Geometry check sheet. Reference: the model listing, model coordinates, mm. Face numbers are marked on the shaded views. Round coordinates to 2 decimals unless told otherwise and drop trailing zeros. Loops run counter-clockwise (first coordinate to the right, second up) from the corner with the lowest first, then second, coordinate; pieces in that order, holes last. Notation, with made-up numbers: (11.5, 37.25) -> (29.5, 37.25) arc R7 cw to (29.5, 47.25) -> close; hole circle Ø10 at (18.25, -20.75). An arc over 180 degrees is marked (long way). Use one line per item in the form item = value.
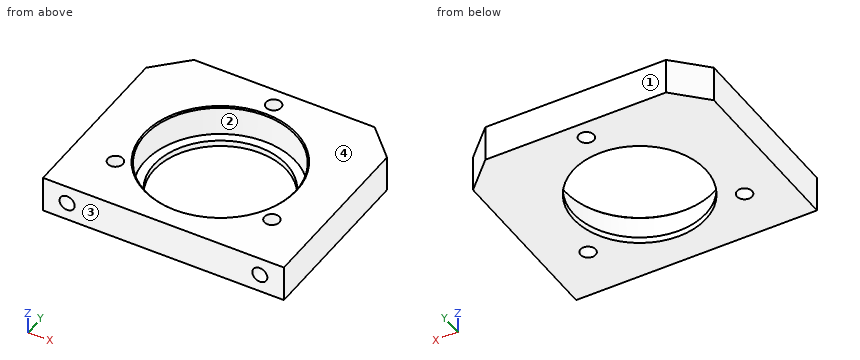
from build123d import *

# Parameters (mm, degrees)
SKETCH_1_R             = 11
EXTRUDE_1_DEPTH        = 6
SKETCH_2_R             = 12.5
CUT_EXTRUDE_1_DEPTH    = 5
HOLE_WIZARD_M3_1_D     = 2.5
HOLE_WIZARD_M3_2_D     = 2.5
HOLE_WIZARD_M3_2_DEPTH = 6
HOLE_WIZARD_M3_2_TIP   = 0.751075774
CHAMFER_1_SIZE         = 0.2


with BuildPart() as part:
    # 草图1 → 凸台-拉伸1 (new body)
    with BuildSketch(Plane.XY):
        Polygon((-20, -16), (20, -16), (20, 13), (15, 18), (-15, 18), (-20, 13), align=None)
        Circle(SKETCH_1_R, mode=Mode.SUBTRACT)
    extrude(amount=EXTRUDE_1_DEPTH)

    # 草图2 → 切除-拉伸1 (cut)
    with BuildSketch(Plane.XY.offset(6)):
        Circle(SKETCH_2_R)
    extrude(amount=-CUT_EXTRUDE_1_DEPTH, mode=Mode.SUBTRACT)

    # M3 螺纹孔1 (through all)
    with Locations(Plane(origin=(0, 15.005632156, 6), x_dir=(1, 0, 0), z_dir=(0, 0, 1))):
        with Locations((0, 0), (-12.990381057, -22.505632156), (12.990381057, -22.505632156)):
            Hole(HOLE_WIZARD_M3_1_D / 2)

    # M3 螺纹孔2
    with Locations(Plane(origin=(-16, -16, 3), x_dir=(0, 0, -1), z_dir=(0, -1, 0))):
        with Locations((0, 0), (0, 32)):
            Hole(HOLE_WIZARD_M3_2_D / 2, depth=HOLE_WIZARD_M3_2_DEPTH)
            with Locations((0, 0, -(HOLE_WIZARD_M3_2_DEPTH + HOLE_WIZARD_M3_2_TIP / 2))):  # 118° drill point
                Cone(0, HOLE_WIZARD_M3_2_D / 2, HOLE_WIZARD_M3_2_TIP, mode=Mode.SUBTRACT)

    # 倒角1
    chamfer_1_edges = [part.edges().sort_by_distance(p)[0] for p in [
        (-12.5, 0, 6),
    ]]
    chamfer(chamfer_1_edges, length=CHAMFER_1_SIZE)


solid = part.part
1. Gauge pin test, flat ends, axial feed: pin 1 (2 mm diameter, centred on x = -16, z = 3, fed in from -Y); pin 2 (1.5 mm diameter, centred on x = 16, z = 3, fed in from +Y). Record the tip position at first contact, or that the pin passes through.
Return value:
pin_1 = -9.85
pin_2 = 17.75
2. Section check A-A (z = 5.35). Record the boundary of the cut face in (x, y), then the cut area to 3 significant figures.
Return value:
outline = (-20, -16) -> (20, -16) -> (20, 13) -> (15, 18) -> (-15, 18) -> (-20, 13) -> close; hole circle Ø2.5 at (-12.99, -7.5); hole circle Ø25 at (0, 0); hole circle Ø2.5 at (0, 15.01); hole circle Ø2.5 at (12.99, -7.5)
area = 829 mm2
3. Section check C-C (z = 0.45). Record the boundary of the cut face in (x, y), then the cut area to 3 significant figures.
Return value:
outline = (-20, -16) -> (20, -16) -> (20, 13) -> (15, 18) -> (-15, 18) -> (-20, 13) -> close; hole circle Ø2.5 at (-12.99, -7.5); hole circle Ø22 at (0, 0); hole circle Ø2.5 at (0, 15.01); hole circle Ø2.5 at (12.99, -7.5)
area = 940 mm2
4. Section check B-B (y = -7.5). Count the separate pieces of the cut face and the enclosed holes in it, then the cut area to 3 significant figures.
Return value:
separate_pieces = 4
enclosed_holes = 0
area = 93.9 mm2
5. Mould release check, pull along Y, two halves, no side actions. Record for the marked faces 1, 2, 3 and 4: released by +Y, released by -Y, zero draft, split by the parting line, or undercut.
Return value:
face_1 = released by +Y
face_2 = undercut
face_3 = released by -Y
face_4 = zero draft
6. Material ranges on line 1 along Y through (x, z) = (0, 0.4); line 2 along Y through (x, z) = (0, 2.7); line 3 along Z through (x, y) = (16, -11.5), recorded low to high.
Return value:
line_1 = -16 to -11, 11 to 13.76, 16.26 to 18
line_2 = -16 to -12.5, 12.5 to 13.76, 16.26 to 18
line_3 = 0 to 1.75, 4.25 to 6
